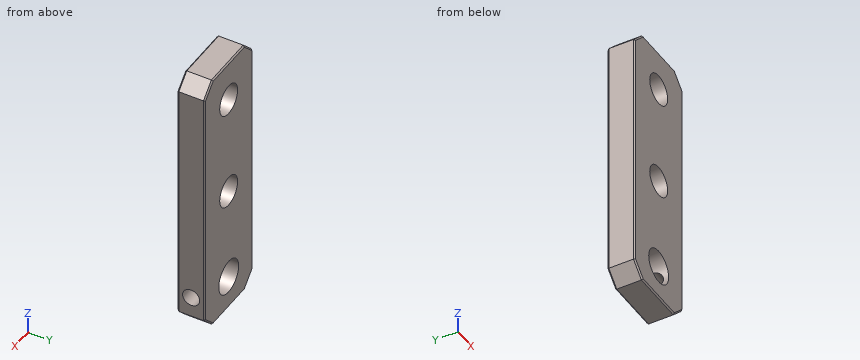
from build123d import *

# Parameters (mm, degrees)
SKETCH1_W                  = 12
SKETCH1_H                  = 40
BOSS_EXTRUDE1_DEPTH        = 2
CHAMFER1_SIZE              = 2
M6_TAPPED_HOLE1_D          = 5
F_4_5_4_5_DIAMETER_HOLE1_D = 4.5
M3_TAPPED_HOLE1_REACH      = 25.409
M3_TAPPED_HOLE1_BORE_R     = 1.25
CHAMFER2_SIZE              = 0.2


with BuildPart() as part:
    # Sketch1 → Boss-Extrude1 (new, symmetric)
    with BuildSketch(Plane(origin=(0, 0, 0), x_dir=(1, 0, 0), z_dir=(0, 1, 0))):
        Rectangle(SKETCH1_W, SKETCH1_H)
    extrude(amount=BOSS_EXTRUDE1_DEPTH, both=True)

    # Chamfer1
    chamfer1_edges = [part.edges().sort_by_distance(p)[0] for p in [
        (6, 0, 20),
        (-6, 0, 20),
        (-6, 0, -20),
        (6, 0, -20),
    ]]
    chamfer(chamfer1_edges, length=CHAMFER1_SIZE)

    # M6 Tapped Hole1 (through all)
    with Locations(Plane(origin=(0, 2, 0), x_dir=(1, 0, 0), z_dir=(0, 1, 0))):
        with Locations((0, 15)):
            Hole(M6_TAPPED_HOLE1_D / 2)

    # Ø4.5 (4.5) Diameter Hole1 (through all)
    with Locations(Plane(origin=(0, 2, 0), x_dir=(1, 0, 0), z_dir=(0, 1, 0))):
        with Locations((0, 1), (0, -14)):
            Hole(F_4_5_4_5_DIAMETER_HOLE1_D / 2)

    # M3 Tapped Hole1 bore → M3 Tapped Hole1 (cut, up to next)
    with BuildSketch(Plane(origin=(6, 0, 0), x_dir=(0, 0, -1), z_dir=(1, 0, 0)), mode=Mode.PRIVATE) as m3_tapped_hole1_sk1:
        with Locations((15, 0)):
            Circle(M3_TAPPED_HOLE1_BORE_R)
    m3_tapped_hole1_tool1 = extrude(m3_tapped_hole1_sk1.sketch, amount=-M3_TAPPED_HOLE1_REACH, mode=Mode.PRIVATE) & part.part
    add(m3_tapped_hole1_tool1.solids().sort_by_distance((6, 0, -15))[0], mode=Mode.SUBTRACT)

    # Chamfer2
    chamfer2_edges = [part.edges().sort_by_distance(p)[0] for p in [
        (-6, -2, 0),
        (-6, 2, 0),
        (6, -2, 0),
        (0, -2, 20),
        (0, -2, -20),
        (-5, -2, 19),
        (5, -2, 19),
        (5, -2, -19),
        (-5, -2, -19),
        (0, 2, -20),
        (6, 2, 0),
        (0, 2, 20),
        (-5, 2, 19),
        (5, 2, 19),
        (5, 2, -19),
        (-5, 2, -19),
    ]]
    chamfer(chamfer2_edges, length=CHAMFER2_SIZE)


solid = part.part
CAD build for the part. Positions are in the model's coordinates, mm. Round coordinates to 2 decimals unless told otherwise and drop trailing zeros. Write each loop counter-clockwise with the first axis right and the second up, starting at its lowest first coordinate (ties: lowest second). Pieces come first, ordered by that corner, then holes.
(1) Slice it at C-C, the plane y = 0. Write the cut outline in (x, z), and give its area (3 significant figures).
(2) Slice it at D-D, the plane z = -15. Write the cut outline in (x, y).
(3) Probe line 1 along Z through (x, y) = (0, 0.85); line 2 along Z through (x, y) = (-1.5, -1.05); line 3 along Y through (x, z) = (4, -15). List the from-to ranges inside material, lowest first.
(4) Slice it at B-B, the plane x = 0. Write the cut outline in (y, z), and give its area (3 significant figures).
(5) Drop a flat-ended pin along its axis: P1, Ø5, axis at x = 0, z = -1, coming from the +Y side. Give the stop position or say it passes through.
(6) Slice it at A-A, the plane z = 14. Write the cut outline in (x, y).
From the geometry:
1. outline: (-6, -18) - (-4, -20) - (4, -20) - (6, -18) - (6, -16.25) - (2.17, -16.25) arc R2.5 cw (long way) to (2.17, -13.75) - (6, -13.75) - (6, 18) - (4, 20) - (-4, 20) - (-6, 18) - close; hole circle Ø4.5 at (0, -1); hole circle Ø4.5 at (0, 14)
1. area: 412 mm2
2. outline: (-6, -1.8) - (-5.8, -2) - (-2.5, -2) - (-2.5, 2) - (-5.8, 2) - (-6, 1.8) - close; (2.5, -2) - (5.8, -2) - (6, -1.8) - (6, -1.25) - (2.5, -1.25) - close; (2.5, 1.25) - (6, 1.25) - (6, 1.8) - (5.8, 2) - (2.5, 2) - close
3. line 1: z = -20 to -17.5, -12.5 to -3.25, 1.25 to 11.75, 16.25 to 20
3. line 2: z = -20 to -17, -13 to -2.68, 0.68 to 12.32, 15.68 to 20
3. line 3: y = -2 to -1.25, 1.25 to 2
4. outline: (-2, -19.8) - (-1.8, -20) - (1.8, -20) - (2, -19.8) - (2, -17.5) - (-2, -17.5) - close; (-2, -12.5) - (2, -12.5) - (2, -3.25) - (-2, -3.25) - close; (-2, 1.25) - (2, 1.25) - (2, 11.75) - (-2, 11.75) - close; (-2, 16.25) - (2, 16.25) - (2, 19.8) - (1.8, 20) - (-1.8, 20) - (-2, 19.8) - close
4. area: 104 mm2
5. P1: stops at y = 2
6. outline: (-6, -1.8) - (-5.8, -2) - (-2.25, -2) - (-2.25, 2) - (-5.8, 2) - (-6, 1.8) - close; (2.25, -2) - (5.8, -2) - (6, -1.8) - (6, 1.8) - (5.8, 2) - (2.25, 2) - close
